from build123d import *

# Parameters (mm, degrees)
BASE_BLOCK_DEPTH       = 22
LUG_WEB_SKETCH_W       = 20
LUG_WEB_SKETCH_H       = 44
LUG_WEB_DEPTH          = 24
LUG_BOSS_1_SKETCH_R    = 22
LUG_BOSS_1_SKETCH_R_2  = 11
LUG_BOSS_1_R22_DEPTH   = 20
LUG_HOLE_1_SKETCH_R    = 11
LUG_HOLE_1_DEPTH       = 20
LUG_START              = -20
LUG_BOSS_2_SKETCH_R    = 22
LUG_BOSS_2_SKETCH_R_2  = 11
LUG_BOSS_2_R22_DEPTH   = 20
LUG_HOLE_2_SKETCH_R    = 11
LUG_HOLE_2_DEPTH       = 20
CLEVIS_SLOT_DEPTH      = 73.828565824
CLEVIS_SLOT_DEPTH_BACK = 20


with BuildPart() as part:
    # Base Profile Sketch → Base Block (new, symmetric)
    with BuildSketch(Plane.XY):
        Polygon((-36, 0), (36, 0), (36, 32), (16, 32), (16, 12), (-36, 12), align=None)
    extrude(amount=BASE_BLOCK_DEPTH, both=True)

    # Lug Web Sketch → Lug Web (add)
    with BuildSketch(Plane.XZ):
        with Locations((-26, 0)):
            Rectangle(LUG_WEB_SKETCH_W, LUG_WEB_SKETCH_H)
        with Locations((26, 0)):
            Rectangle(LUG_WEB_SKETCH_W, LUG_WEB_SKETCH_H)
    extrude(amount=LUG_WEB_DEPTH)

    # Lug Boss 1 Sketch → Lug Boss 1 R22 (add)
    with BuildSketch(Plane.ZY.offset(36)):
        with Locations((0, -24)):
            Circle(LUG_BOSS_1_SKETCH_R)
        with Locations((0, -24)):
            Circle(LUG_BOSS_1_SKETCH_R_2, mode=Mode.SUBTRACT)
    extrude(amount=-LUG_BOSS_1_R22_DEPTH)

    # Lug Hole 1 Sketch → Lug Hole 1 (cut)
    with BuildSketch(Plane.ZY.offset(36)):
        with Locations(Location((0, -24, 0), (0, 0, 270))):
            Circle(LUG_HOLE_1_SKETCH_R)
    extrude(amount=-LUG_HOLE_1_DEPTH, mode=Mode.SUBTRACT)

    # Lug Boss 2 Sketch → Lug Boss 2 R22 (add)
    with BuildSketch(Plane(origin=(36, 0, 0), x_dir=(0, 0, -1), z_dir=(1, 0, 0)).offset(LUG_START)):
        with Locations((0, -24)):
            Circle(LUG_BOSS_2_SKETCH_R)
        with Locations(Location((0, -24, 0), (0, 0, 270))):
            Circle(LUG_BOSS_2_SKETCH_R_2, mode=Mode.SUBTRACT)
    extrude(amount=LUG_BOSS_2_R22_DEPTH)

    # Lug Hole 2 Sketch → Lug Hole 2 (cut)
    with BuildSketch(Plane(origin=(36, 0, 0), x_dir=(0, 0, -1), z_dir=(1, 0, 0)).offset(LUG_START)):
        with Locations(Location((0, -24, 0), (0, 0, 270))):
            Circle(LUG_HOLE_2_SKETCH_R)
    extrude(amount=LUG_HOLE_2_DEPTH, mode=Mode.SUBTRACT)

    # Clevis Slot Sketch → Clevis Slot (cut, two sides: drawn at the far end of the back side and taken through both)
    with BuildSketch(Plane.ZY.offset(-16).offset(-CLEVIS_SLOT_DEPTH_BACK)):
        with BuildLine():
            Line((-10, 32), (-10, 24))
            ThreePointArc((-10, 24), (0, 14), (10, 24))
            Line((10, 24), (10, 32))
            Line((10, 32), (-10, 32))
        make_face()
    extrude(amount=CLEVIS_SLOT_DEPTH + CLEVIS_SLOT_DEPTH_BACK, mode=Mode.SUBTRACT)


solid = part.part
Check sheet for the modelled part. Datum: model origin and axes. Units: mm. A direction names the side the tool comes from. Round coordinates to 2 decimals unless told otherwise and drop trailing zeros. Loops run counter-clockwise (first coordinate to the right, second up) from the corner with the lowest first, then second, coordinate; pieces in that order, holes last. Notation, with made-up numbers: (69.25, -32.5) - (80.25, -32.5) arc R21 cw to (80.25, -21.5) - close; hole circle Ø5 at (48.25, 1). An arc over 180 degrees is marked (long way). Answer as CSV lines item,"result". Start each with the question number.
Item 1: Section check C-C (y = -19.5). Record the boundary of the cut face in (x, z), and give its area (3 significant figures).
Item 2: Set-up check for faces 1 (the flat face through (26, 28, -10)), 2 (the flat face through (16, -12, 0)), 3 (the flat face through (16, 13, 0)): record each of +Z, -Z, +X, -X, +Y, -Y from which the full face is reachable in a straight line by a thin tool's end or side.
Item 3: Section check A-A (x = 19). Record the boundary of the cut face in (y, z).
Item 4: Section check D-D (y = 20). Record the boundary of the cut face in (x, z).
Item 5: Scan lines: line 1 (Z direction, x = -28.75, y = -24); line 2 (X direction, y = -38.5, z = -12.5); line 3 (Y direction, x = -24.75, z = 0). Record each from-to range of solid material in increasing order. Write a range as [from, to].
Item 6: Depth check by flat-ended pin: P1, Ø1, axis at x = 28, z = -7, coming from the +Y side; P2, Ø8, axis at x = -26, z = -8.5, coming from the -Y side; P3, Ø10, axis at y = 17.5, z = 1, coming from the -X side; P4, Ø17.5, axis at y = -24, z = 0, coming from the -X side. Enter the tip coordinate at first touch or a pass-through.
Item 7: Section check B-B (z = 0). Record the boundary of the cut face in (x, y), and give its area (3 significant figures).
Item 8: Release check for a two-part mould opening along Y. For faces 4 (the cylindrical face through (25.86, -33.759, -5.076)), 5 (the flat face through (-1, 4, -22)), 6 (the cylindrical face through (26, -46, 0)), 7 (the cylindrical face through (-26.14, -34.74, -2.38)) record: +Y half, -Y half, draft (parallel to the pull), parting line (faces both ways), or undercut.
Report:
1,outline,"(-36, -22) - (-16, -22) - (-16, -10.04) - (-36, -10.04) - close; (-36, 10.04) - (-16, 10.04) - (-16, 22) - (-36, 22) - close; (16, -22) - (36, -22) - (36, -10.04) - (16, -10.04) - close; (16, 10.04) - (36, 10.04) - (36, 22) - (16, 22) - close"
1,area,"957 mm2"
2,face 1,"+X, -X, +Y"
2,face 2,"+Z, -Z, -Y"
2,face 3,"+Z, -Z, -X, +Y"
3,outline,"(-24, -22) - (32, -22) - (32, -10) - (24, -10) arc R10 cw to (24, 10) - (32, 10) - (32, 22) - (-24, 22) arc R22 ccw to start; hole circle Ø22 at (-24, 0)"
4,outline,"(16, -22) - (36, -22) - (36, -9.17) - (16, -9.17) - close; (16, 9.17) - (36, 9.17) - (36, 22) - (16, 22) - close"
5,line 1,"z = [-22, -11], [11, 22]"
5,line 2,"x = [-36, -16], [16, 36]"
5,line 3,"y = [-46, -35], [-13, 12]"
6,P1,"stops at y = 17.39"
6,P2,"stops at y = -45.53"
6,P3,"stops at x = 16"
6,P4,"passes through"
7,outline,"(-36, -46) - (-16, -46) - (-16, -35) - (-36, -35) - close; (-36, -13) - (-16, -13) - (-16, 0) - (16, 0) - (16, -13) - (36, -13) - (36, 14) - (16, 14) - (16, 12) - (-36, 12) - close; (16, -46) - (36, -46) - (36, -35) - (16, -35) - close"
7,area,"1,860 mm2"
8,face 4,"undercut"
8,face 5,"draft"
8,face 6,"-Y half"
8,face 7,"undercut"
